from build123d import *

# Parameters (mm, degrees)
EXTRUDE_THIN1_DEPTH = 50
SKETCH2_R           = 3.5
CUT_EXTRUDE1_DEPTH  = 953.351825745
CUT_EXTRUDE2_DEPTH  = 954.456868453
CUT_EXTRUDE3_DEPTH  = 951.073377733
CUT_EXTRUDE4_DEPTH  = 954.344114158
FILLET1_R           = 2


with BuildPart() as part:
    # Sketch1 → Extrude-Thin1 (new, symmetric)
    with BuildSketch(Plane.XY):
        Polygon((0, 0), (495, 0), (945, 90), (945, 107), (946, 107), (946, 89.180196097), (495.099019514, -1), (0, -1), align=None)
    extrude(amount=EXTRUDE_THIN1_DEPTH, both=True)

    # Sketch2 → Cut-Extrude1 (cut, through all)
    with BuildSketch(Plane.ZY.offset(-945)):
        with Locations((-44, 100)):
            Circle(SKETCH2_R)
        with Locations((44, 100)):
            Circle(SKETCH2_R)
    extrude(amount=-CUT_EXTRUDE1_DEPTH, mode=Mode.SUBTRACT)

    # Sketch3 → Cut-Extrude2 (cut, through all)
    with BuildSketch(Plane.XZ.offset(1)):
        with BuildLine():
            Line((42.5, 46.5), (47.5, 46.5))
            ThreePointArc((47.5, 46.5), (50, 44), (47.5, 41.5))
            Line((47.5, 41.5), (42.5, 41.5))
            ThreePointArc((42.5, 41.5), (40, 44), (42.5, 46.5))
        make_face()
        with BuildLine():
            Line((42.5, -41.5), (47.5, -41.5))
            ThreePointArc((47.5, -41.5), (50, -44), (47.5, -46.5))
            Line((47.5, -46.5), (42.5, -46.5))
            ThreePointArc((42.5, -46.5), (40, -44), (42.5, -41.5))
        make_face()
        with BuildLine():
            Line((392.5, -41.5), (397.5, -41.5))
            ThreePointArc((397.5, -41.5), (400, -44), (397.5, -46.5))
            Line((397.5, -46.5), (392.5, -46.5))
            ThreePointArc((392.5, -46.5), (390, -44), (392.5, -41.5))
        make_face()
        with BuildLine():
            Line((392.5, 46.5), (397.5, 46.5))
            ThreePointArc((397.5, 46.5), (400, 44), (397.5, 41.5))
            Line((397.5, 41.5), (392.5, 41.5))
            ThreePointArc((392.5, 41.5), (390, 44), (392.5, 46.5))
        make_face()
    extrude(amount=-CUT_EXTRUDE2_DEPTH, mode=Mode.SUBTRACT)

    # Sketch4 → Cut-Extrude3 (cut, through all)
    with BuildSketch(Plane(origin=(19.038461538, -95.192307692, 0), x_dir=(0.9805806756909202, 0.1961161351381841, 0), z_dir=(-0.1961161351381841, 0.9805806756909202, 0))):
        with BuildLine():
            Line((541.79919069, 46.5), (546.79919069, 46.5))
            ThreePointArc((546.79919069, 46.5), (549.29919069, 44), (546.79919069, 41.5))
            Line((546.79919069, 41.5), (541.79919069, 41.5))
            ThreePointArc((541.79919069, 41.5), (539.29919069, 44), (541.79919069, 46.5))
        make_face()
        with BuildLine():
            Line((541.79919069, -41.5), (546.79919069, -41.5))
            ThreePointArc((546.79919069, -41.5), (549.29919069, -44), (546.79919069, -46.5))
            Line((546.79919069, -46.5), (541.79919069, -46.5))
            ThreePointArc((541.79919069, -46.5), (539.29919069, -44), (541.79919069, -41.5))
        make_face()
        with BuildLine():
            Line((891.79919069, -41.5), (896.79919069, -41.5))
            ThreePointArc((896.79919069, -41.5), (899.29919069, -44), (896.79919069, -46.5))
            Line((896.79919069, -46.5), (891.79919069, -46.5))
            ThreePointArc((891.79919069, -46.5), (889.29919069, -44), (891.79919069, -41.5))
        make_face()
        with BuildLine():
            Line((891.79919069, 46.5), (896.79919069, 46.5))
            ThreePointArc((896.79919069, 46.5), (899.29919069, 44), (896.79919069, 41.5))
            Line((896.79919069, 41.5), (891.79919069, 41.5))
            ThreePointArc((891.79919069, 41.5), (889.29919069, 44), (891.79919069, 46.5))
        make_face()
    extrude(amount=-CUT_EXTRUDE3_DEPTH, mode=Mode.SUBTRACT)

    # Sketch5 → Cut-Extrude4 (cut, through all)
    with BuildSketch(Plane(origin=(0, 0, 0), x_dir=(1, 0, 0), z_dir=(0, 1, 0))):
        with BuildLine():
            Line((0, -25), (40, -25))
            ThreePointArc((40, -25), (65, 0), (40, 25))
            Line((40, 25), (0, 25))
            Line((0, 25), (0, -25))
        make_face()
    extrude(amount=-CUT_EXTRUDE4_DEPTH, mode=Mode.SUBTRACT)

    # Fillet1
    fillet1_edges = [part.edges().sort_by_distance(p)[0] for p in [
        (946, 89.180196097, 0),
        (495.099019514, -1, 0),
        (495, 0, 0),
        (945, 90, 0),
        (0, -0.5, 25),
        (0, -0.5, -25),
        (0, -0.5, 50),
        (945.5, 107, 50),
        (0, -0.5, -50),
        (945.5, 107, -50),
    ]]
    fillet(fillet1_edges, radius=FILLET1_R)


solid = part.part
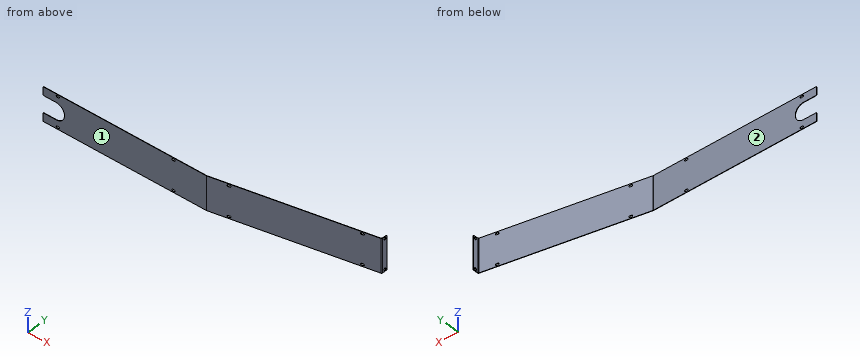
Verification items for the finished model (mm, model axes). Face numbers are marked on the shaded views. A direction names the side the tool comes from. Give positions to 0.01 mm unless a question says otherwise; leave off trailing zeros. Write each loop counter-clockwise with the first axis right and the second up, starting at its lowest first coordinate (ties: lowest second). Pieces come first, ordered by that corner, then holes. Notation, with made-up numbers: M 60,47 L 93,47 A30 cw 93,78 Z; hole C 52.5,44 d4. An arc over 180 degrees is marked long. Put each result on its own line as item: value. Start each with the question number.
1. Section check C-C (y = 31). Record the cut outline in (x, z), and give its area (3 significant figures).
2. Set-up check for the marked faces 1 and 2: record each of +Z, -Z, +X, -X, +Y, -Y from which the full face is reachable in a straight line by a thin tool's end or side.
3. Go/stop test with flat-tipped pins: pin 1 Ø1 at (x, z) = (553.5, -39.5) entering from -Y; pin 2 Ø2 at (x, z) = (664, 2) entering from +Y; pin 3 Ø7.5 at (y, z) = (97, -17) entering from -X. Record where each tip stops, or that it passes through.
4. Section check A-A (z = 0). Record the cut outline in (x, y).
5. Scan lines: line 1 along Y through (x, z) = (301, -33); line 2 along X through (y, z) = (93, 22.5); line 3 along Y through (x, z) = (945.45, -44). Record each from-to range of solid material in increasing order. Write a range as [from, to].
6. Section check B-B (x = 415). Record the cut outline in (y, z).
Answer list:
1. outline: M 650,-50 L 655.1,-50 L 655.1,50 L 650,50 Z
1. area: 510 mm2
2. face 1: +Z, -Z, +X, -X, -Y
2. face 2: +Z, -Z, -X, +Y
3. pin 1: y = 10.58
3. pin 2: y = 34
3. pin 3: x = 945
4. outline: M 65,-1 L 494.9,-1 A2 ccw 495.29,-0.96 L 944.39,88.86 A2 ccw 946,90.82 L 946,107 L 945,107 L 945,91.64 A2 cw 943.39,89.68 L 495.19,0.04 A2 cw 494.8,0 L 65,0 Z
5. line 1: [-1, 0]
5. line 2: [945, 946]
5. line 3: [89.44, 96.5], [103.5, 107]
6. outline: M -1,-50 L 0,-50 L 0,50 L -1,50 Z
